```python
from build123d import *

# Parameters (mm, degrees)
BOSS_EXTRUDE1_DEPTH = 45
SKETCH2_R           = 8
CUT_EXTRUDE1_DEPTH  = 153.358130732


with BuildPart() as part:
    # Sketch1 → Boss-Extrude1 (new body)
    with BuildSketch(Plane.XY):
        with BuildLine():
            Line((0, 0), (0, -137))
            ThreePointArc((0, -137), (1.464466094, -140.535533906), (5, -142))
            Line((5, -142), (27, -142))
            ThreePointArc((27, -142), (30.535533906, -140.535533906), (32, -137))
            Line((32, -137), (32, 0))
            Line((32, 0), (29, 0))
            Line((29, 0), (29, -137))
            ThreePointArc((29, -137), (28.414213562, -138.414213562), (27, -139))
            Line((27, -139), (5, -139))
            ThreePointArc((5, -139), (3.585786438, -138.414213562), (3, -137))
            Line((3, -137), (3, 0))
            Line((3, 0), (0, 0))
        make_face()
    extrude(amount=BOSS_EXTRUDE1_DEPTH)

    # Sketch2 → Cut-Extrude1 (cut, through all)
    with BuildSketch(Plane(origin=(32, 0, 0), x_dir=(0, 0, -1), z_dir=(1, 0, 0))):
        with Locations((-22.5, -12)):
            Circle(SKETCH2_R)
    extrude(amount=-CUT_EXTRUDE1_DEPTH, mode=Mode.SUBTRACT)


solid = part.part
```
Verification items for the finished model (mm, model axes). A direction names the side the tool comes from. Coordinates: 2 decimals unless noted, no trailing zeros. Write each loop counter-clockwise with the first axis right and the second up, starting at its lowest first coordinate (ties: lowest second). Pieces come first, ordered by that corner, then holes. Notation, with made-up numbers: M 5.25,81.25 L 41.25,81.25 A11 cw 41.25,87.25 Z; hole C 80,-32 d5. An arc over 180 degrees is marked long. Answer as a JSON object with one key per item and string values. Group by question number.
(1) Cross-section at B-B, the plane z = 22.5. Record the cut outline in (x, y).
(2) Cross-section at C-C, the plane y = -28. Record the cut outline in (x, z).
(3) Release check for a two-part mould opening along Y. For faces 1 (the face through (0, -68, 22)), 2 (the face through (1.521, -16.868, 28.849)), 3 (the face through (16, -139, 22)) record: +Y half, -Y half, draft (parallel to the pull), parting line (faces both ways), or undercut.
(4) Tool access check on faces 4 (the face through (29, -68, 22)), 5 (the face through (30, -141, 22)). Record the directions out of +Z, -Z, +X, -X, +Y, -Y that give a thin tool (end or side, any length) a straight path to the whole face; none if there is none.
(5) Cross-section at A-A, the plane y = -12. Record the cut outline in (x, z), and give its area (3 significant figures).
(6) Cross-section at D-D, the plane x = 23. Record the cut outline in (y, z).
(7) Material ranges on line 1 (X direction, y = -54, z = 9.5); line 2 (Y direction, x = 7, z = 37); line 3 (Y direction, x = 31.35, z = 22.5), recorded low to high.
(8) Gauge pin test, flat ends, axial feed: pin 1 (2 mm diameter, centred on x = 12.5, z = 20.5, fed in from +Y); pin 2 (9.5 mm diameter, centred on y = -12, z = 22.5, fed in from +X); pin 3 (6 mm diameter, centred on x = 7, z = 20.5, fed in from +Y). Record the tip position at first contact, or that the pin passes through.
Reply:
{
 "1": {"outline": "M 0,-137 A5 ccw 5,-142 L 27,-142 A5 ccw 32,-137 L 32,-20 L 29,-20 L 29,-137 A2 cw 27,-139 L 5,-139 A2 cw 3,-137 L 3,-20 L 0,-20 Z; M 0,-4 L 3,-4 L 3,0 L 0,0 Z; M 29,-4 L 32,-4 L 32,0 L 29,0 Z"},
 "2": {"outline": "M 0,0 L 3,0 L 3,45 L 0,45 Z; M 29,0 L 32,0 L 32,45 L 29,45 Z"},
 "3": {"face 1": "draft", "face 2": "undercut", "face 3": "+Y half"},
 "4": {"face 4": "+Z, -Z, +Y", "face 5": "+Z, -Z, +X, -Y"},
 "5": {"outline": "M 0,0 L 3,0 L 3,14.5 L 0,14.5 Z; M 0,30.5 L 3,30.5 L 3,45 L 0,45 Z; M 29,0 L 32,0 L 32,14.5 L 29,14.5 Z; M 29,30.5 L 32,30.5 L 32,45 L 29,45 Z", "area": "174 mm²"},
 "6": {"outline": "M -142,0 L -139,0 L -139,45 L -142,45 Z"},
 "7": {"line 1": "0 to 3, 29 to 32", "line 2": "-142 to -139", "line 3": "-139.47 to -20, -4 to 0"},
 "8": {"pin 1": "y = -139", "pin 2": "through", "pin 3": "y = -138.73"}
}
